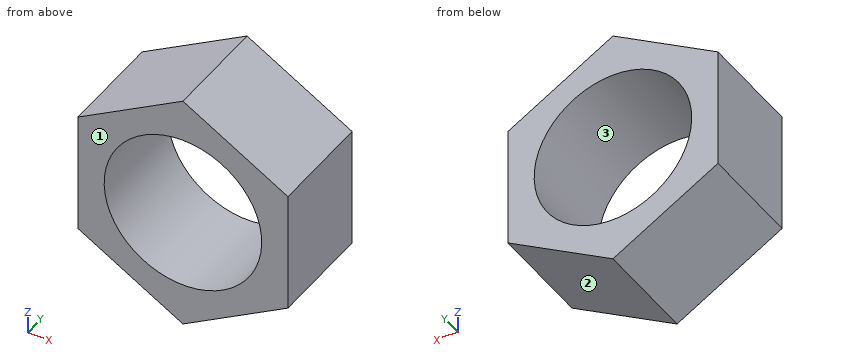
from build123d import *

# Parameters (mm, degrees)
HEX_PROFILE_16AF_WITH_BORE_12_R = 6
NUT_BODY_8_MM_DEPTH             = 4


with BuildPart() as part:
    # Hex Profile 16AF with Bore Ø12 → Nut Body 8 mm (new, symmetric)
    with BuildSketch(Plane(origin=(0, 0, 0), x_dir=(1, 0, 0), z_dir=(0, 1, 0))):
        Polygon((0, -9.237604307), (8, -4.618802154), (8, 4.618802154), (0, 9.237604307), (-8, 4.618802154), (-8, -4.618802154), align=None)
        with Locations(Location((0, 0, 0), (0, 0, 270))):
            Circle(HEX_PROFILE_16AF_WITH_BORE_12_R, mode=Mode.SUBTRACT)
    extrude(amount=NUT_BODY_8_MM_DEPTH, both=True)


solid = part.part
Work out the finished part from the listing and answer in its coordinate system (mm). Face numbers are marked on the shaded views. Give positions to 0.01 mm unless a question says otherwise; leave off trailing zeros. Order: outer loops, then holes, each group sorted by start corner. A loop starts at its lowest first (then second) coordinate and runs counter-clockwise, first axis right, second up. Notation, with made-up numbers: (-31, 37) -> (21, 37) arc R32 ccw to (21, 76) -> close; hole circle Ø8 at (37.25, 61). An arc over 180 degrees is marked (long way). One line per item, written item: value.
Item 1: Find section B-B, the plane y = 1.5. Give the vertices of the cut face in (x, z), plus the area to 3 significant figures.
Answer sheet:
outline: (-8, -4.62) -> (0, -9.24) -> (8, -4.62) -> (8, 4.62) -> (0, 9.24) -> (-8, 4.62) -> close; hole circle Ø12 at (0, 0)
area: 109 mm²
Item 2: A flat-ended cylindrical pin translates along its axis: P1, Ø1, axis at x = -1.5, y = -1, coming from the +Z side. Find the tip coordinate at first contact, or state that the pin passes through.
Answer sheet:
P1: z = 8.66
Item 3: Straight lines are drawn through the part: probe 1 along X at (y, z) = (0, 0); probe 2 along Z at (x, y) = (-4, -2.5); probe 3 along Z at (x, y) = (3.5, -1.5). For each, find the intervals that lie inside material, in ascending order.
Answer sheet:
probe 1: -8 to -6, 6 to 8
probe 2: -6.93 to -4.47, 4.47 to 6.93
probe 3: -7.22 to -4.87, 4.87 to 7.22
Item 4: Determine the mould class of the marked faces 1, 2 and 3 for opening direction Z: released by +Z, released by -Z, zero draft, split by the parting line, or undercut.
Answer sheet:
face 1: zero draft
face 2: released by -Z
face 3: undercut
Item 5: Find section D-D, the plane x = 6.75. Give the vertices of the cut face in (y, z).
Answer sheet:
outline: (-4, -5.34) -> (4, -5.34) -> (4, 5.34) -> (-4, 5.34) -> close
Item 6: Find section A-A, the plane z = 0. Give the vertices of the cut face in (x, y).
Answer sheet:
outline: (-8, -4) -> (-6, -4) -> (-6, 4) -> (-8, 4) -> close; (6, -4) -> (8, -4) -> (8, 4) -> (6, 4) -> close
Item 7: Find section C-C, the plane x = -5. Give the vertices of the cut face in (y, z), plus the area to 3 significant figures.
Answer sheet:
outline: (-4, -6.35) -> (4, -6.35) -> (4, -3.32) -> (-4, -3.32) -> close; (-4, 3.32) -> (4, 3.32) -> (4, 6.35) -> (-4, 6.35) -> close
area: 48.5 mm²
